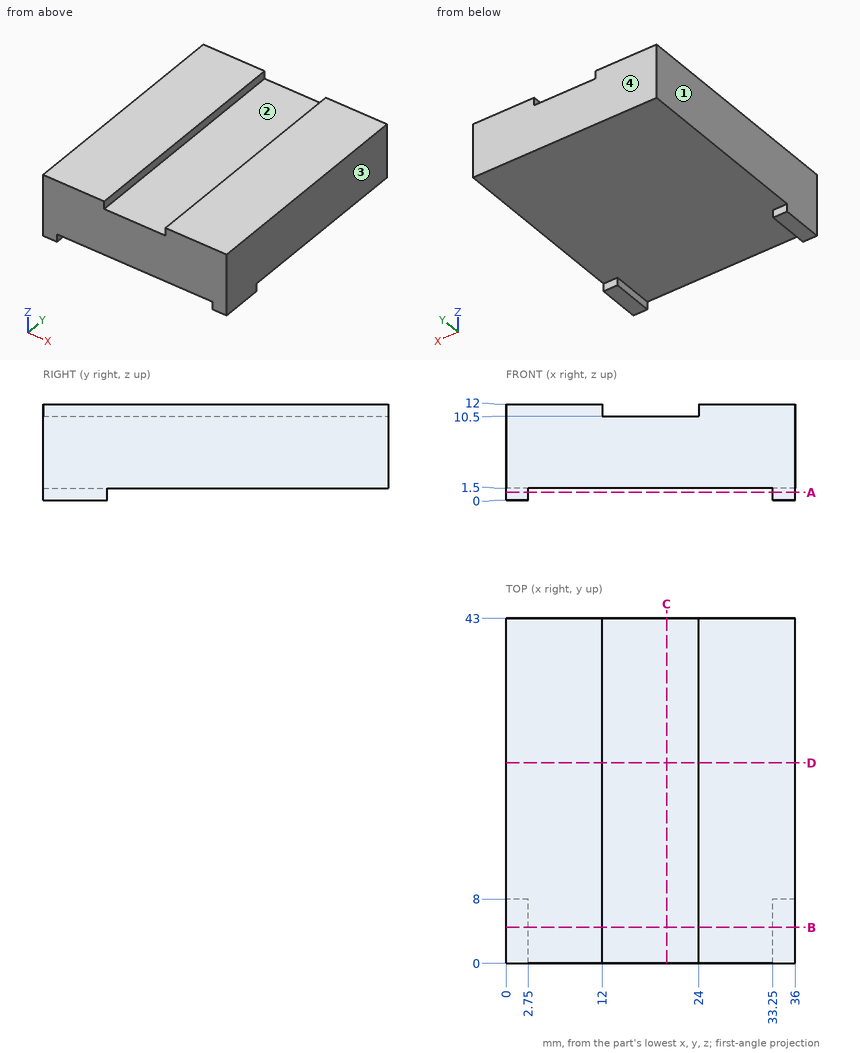
Answer from the drawing. Dimensions are ordinates in mm from the lowest x, y and z of the part. Coordinates: 2 decimals unless noted, no trailing zeros. Write each loop counter-clockwise with the first axis right and the second up, starting at its lowest first coordinate (ties: lowest second). Pieces come first, ordered by that corner, then holes. Notation, with made-up numbers: (16.5, 26) - (35.5, 26) arc R28 ccw to (35.5, 60) - close; hole circle Ø5 at (-31, -19). An arc over 180 degrees is marked (long way). Return JSON: item names as keys, results as strings. Group by question number.
Q1. Find the intervals of material crossed by line 1 along X through (y, z) = (34, 11.25); line 2 along Z through (x, y) = (33.5, 30.5); line 3 along Z through (x, y) = (16.5, 4), in increasing order. Write a range as [from, to].
Q2. The part is cut by section B-B on y = 4.5. Write down the section's boundary in (x, z), and give its area (3 significant figures).
Q3. Flat-ended cylindrical pins translate along their axes: pin 1 Ø5 at (x, y) = (30, 22) entering from -Z; pin 2 Ø1.6 at (x, z) = (2, 0.5) entering from +Y; pin 3 Ø3 at (x, z) = (21, 9.5) entering from -Y; pin 4 Ø9.5 at (x, y) = (17.5, 22.5) entering from +Z. Find the tip coordinate at first contact, or state that the pin passes through.
Q4. The part is cut by section C-C on x = 20. Write down the section's boundary in (y, z), and give its area (3 significant figures).
Q5. The part is cut by section A-A on z = 1. Write down the section's boundary in (x, y).
Q6. For a pull along X with two mould halves and no side action, classify the marked faces 1, 2, 3 and 4 as +X half, -X half, draft (parallel to the pull), parting line (faces both ways), or undercut.
Q7. The part is cut by section D-D on y = 25. Write down the section's boundary in (x, z).
Evaluation:
{
 "1": {"line 1": "x = [0, 12], [24, 36]", "line 2": "z = [1.5, 12]", "line 3": "z = [1.5, 10.5]"},
 "2": {"outline": "(0, 0) - (2.75, 0) - (2.75, 1.5) - (33.25, 1.5) - (33.25, 0) - (36, 0) - (36, 12) - (24, 12) - (24, 10.5) - (12, 10.5) - (12, 12) - (0, 12) - close", "area": "368 mm2"},
 "3": {"pin 1": "stops at z = 1.5", "pin 2": "stops at y = 8", "pin 3": "stops at y = 0", "pin 4": "stops at z = 10.5"},
 "4": {"outline": "(0, 1.5) - (43, 1.5) - (43, 10.5) - (0, 10.5) - close", "area": "387 mm2"},
 "5": {"outline": "(0, 0) - (2.75, 0) - (2.75, 8) - (0, 8) - close; (33.25, 0) - (36, 0) - (36, 8) - (33.25, 8) - close"},
 "6": {"face 1": "-X half", "face 2": "undercut", "face 3": "+X half", "face 4": "draft"},
 "7": {"outline": "(0, 1.5) - (36, 1.5) - (36, 12) - (24, 12) - (24, 10.5) - (12, 10.5) - (12, 12) - (0, 12) - close"}
}
